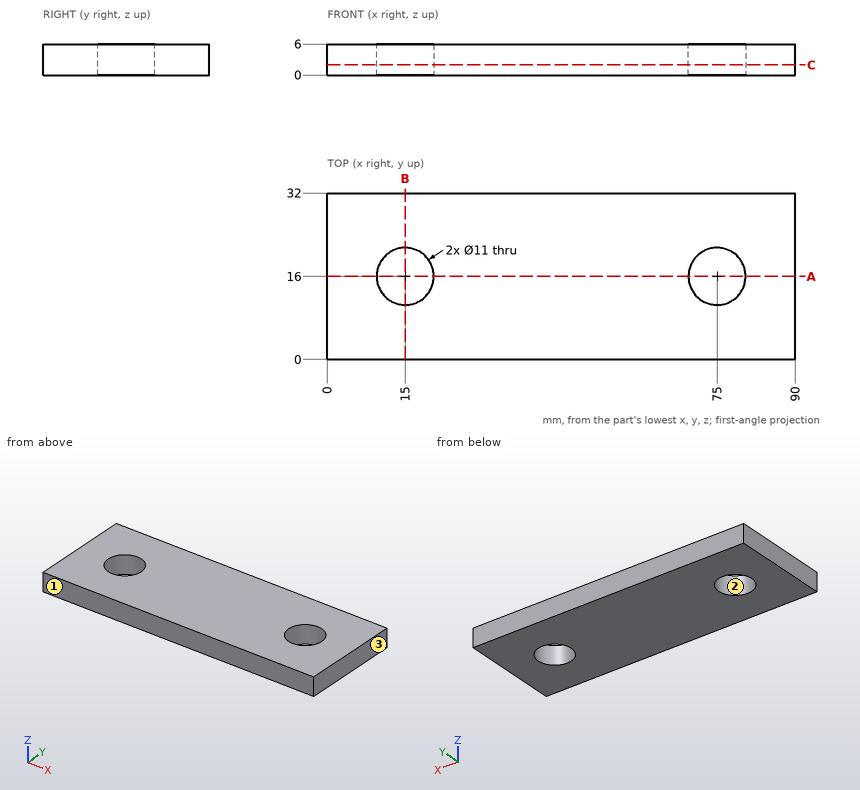
Design review of the part shown in the three views and the two pictorial views. Dimensions are in mm from the part's minimum x, y and z. Give positions to 0.01 mm unless a question says otherwise; leave off trailing zeros. Loops run counter-clockwise (first coordinate to the right, second up) from the corner with the lowest first, then second, coordinate; pieces in that order, holes last. Notation, with made-up numbers: M -4,55 L 19,55 A12 cw 19,60 Z; hole C 40,-26 d1. An arc over 180 degrees is marked long. Write item = value, one per line.
Q1. Draft analysis for pull direction X (two halves, no side actions). For the marked faces 1, 2 and 3, state which applies: +X half, -X half, draft (parallel to the pull), parting line (faces both ways), or undercut.
Output values:
face_1 = draft
face_2 = undercut
face_3 = +X half
Q2. To check wall thickness, follow line 1 (Y direction, x = 15, z = 1.85); line 2 (Y direction, x = 70, z = 1.4). State the ranges of each line that lie inside material, in increasing order. Write a range as [from, to].
Output values:
line_1 = [0, 10.5], [21.5, 32]
line_2 = [0, 13.71], [18.29, 32]
Q3. We need section A-A (y = 16). Give the boundary of the cut face in (x, z).
Output values:
outline = M 0,0 L 9.5,0 L 9.5,6 L 0,6 Z; M 20.5,0 L 69.5,0 L 69.5,6 L 20.5,6 Z; M 80.5,0 L 90,0 L 90,6 L 80.5,6 Z
Q4. Insertion check: pin 1 (1.5 mm diameter, centred on x = 50, y = 12.5, fed in from -Z); pin 2 (10 mm diameter, centred on x = 15, y = 16, fed in from +Z). Each pin has a flat end and moves straight along its axis. Give the tip position at first contact, or say it passes through.
Output values:
pin_1 = 0
pin_2 = through
Q5. We need section C-C (z = 2). Give the boundary of the cut face in (x, y), plus the area to 3 significant figures.
Output values:
outline = M 0,0 L 90,0 L 90,32 L 0,32 Z; hole C 15,16 d11; hole C 75,16 d11
area = 2,690 mm^2
Q6. We need section B-B (x = 15). Give the boundary of the cut face in (y, z), plus the area to 3 significant figures.
Output values:
outline = M 0,0 L 10.5,0 L 10.5,6 L 0,6 Z; M 21.5,0 L 32,0 L 32,6 L 21.5,6 Z
area = 126 mm^2
